from build123d import *

# Parameters (mm, degrees)
SKETCH1_W              = 55
SKETCH1_H              = 20
BOSS_EXTRUDE1_DEPTH    = 25
CHAMFER1_SIZE          = 2
CUT_EXTRUDE1_DEPTH     = 8
HOLE1_D                = 6.6
M12_TAPPED_HOLE1_D     = 10.2
M14X1_5_TAPPED_HOLE1_D = 12.5


with BuildPart() as part:
    # Sketch1 → Boss-Extrude1 (new body)
    with BuildSketch(Plane.XY):
        with Locations((0.549312304, 3.110465116)):
            Rectangle(SKETCH1_W, SKETCH1_H)
    extrude(amount=BOSS_EXTRUDE1_DEPTH)

    # Chamfer1
    chamfer1_edges = [part.edges().sort_by_distance(p)[0] for p in [
        (-26.950687696, 13.110465116, 12.5),
        (28.049312304, 13.110465116, 12.5),
        (28.049312304, -6.889534884, 12.5),
        (-26.950687696, -6.889534884, 12.5),
    ]]
    chamfer(chamfer1_edges, length=CHAMFER1_SIZE)

    # Sketch2 → Cut-Extrude1 (cut)
    with BuildSketch(Plane.XY.offset(25)):
        with BuildLine():
            Line((-21.950687696, 8.610465116), (-26.950687696, 8.610465116))
            Line((-26.950687696, 8.610465116), (-26.950687696, -2.389534884))
            Line((-26.950687696, -2.389534884), (-21.950687696, -2.389534884))
            ThreePointArc((-21.950687696, -2.389534884), (-16.450687696, 3.110465116), (-21.950687696, 8.610465116))
        make_face()
        with BuildLine():
            Line((23.049312304, 8.610465116), (28.049312304, 8.610465116))
            Line((28.049312304, 8.610465116), (28.049312304, -2.389534884))
            Line((28.049312304, -2.389534884), (23.049312304, -2.389534884))
            ThreePointArc((23.049312304, -2.389534884), (17.549312304, 3.110465116), (23.049312304, 8.610465116))
        make_face()
    extrude(amount=-CUT_EXTRUDE1_DEPTH, mode=Mode.SUBTRACT)

    # Hole1 (through all)
    with Locations(Plane.XY.offset(17)):
        with Locations((-21.950687696, 3.110465116), (23.049312304, 3.110465116)):
            Hole(HOLE1_D / 2)

    # M12 Tapped Hole1 (through all)
    with Locations(Plane(origin=(0, -6.889534884, 0), x_dir=(-1, 0, 0), z_dir=(0, -1, 0))):
        with Locations((9.450687696, -12.5)):
            Hole(M12_TAPPED_HOLE1_D / 2)

    # M14x1.5 Tapped Hole1 (through all)
    with Locations(Plane(origin=(0, -6.889534884, 0), x_dir=(-1, 0, 0), z_dir=(0, -1, 0))):
        with Locations((-10.549312304, -12.5)):
            Hole(M14X1_5_TAPPED_HOLE1_D / 2)


solid = part.part
Model file for the job. Use its own axes, mm. A direction names the side the tool comes from. Round coordinates to 2 decimals unless told otherwise and drop trailing zeros. Loops run counter-clockwise (first coordinate to the right, second up) from the corner with the lowest first, then second, coordinate; pieces in that order, holes last. Notation, with made-up numbers: (-22.75, -27.5) - (4.25, -27.5) arc R6 cw to (4.25, -20.5) - close; hole circle Ø10 at (73.5, -28). An arc over 180 degrees is marked (long way). Write each question's results on one line, items separated by ' | '.
(1) Mould opens along Y. For faces 4 (the cylindrical face through (16.323, 3.25, 14.894)), 5 (the flat face through (0, -6.89, 12)), 6 (the flat face through (0, 13.11, 12)), 7 (the cylindrical face through (17.55, 2.99, 21.06)) say: released by +Y, released by -Y, zero draft, split by the parting line, or undercut.
Answer below:
face 4: zero draft | face 5: released by -Y | face 6: released by +Y | face 7: undercut
(2) Wall check: L1, parallel to X at y = 6, z = 11; L2, parallel to X at y = 11, z = 11.5; L3, parallel to X at y = -3, z = 13.75. Give the ranges that are in metal, low to high.
Answer below:
L1: x = -26.95 to -23.54, -20.36 to -14.33, -4.58 to 4.48, 16.62 to 21.46, 24.64 to 28.05 | L2: x = -26.95 to -14.45, -4.45 to 4.38, 16.72 to 28.05 | L3: x = -26.95 to -14.4, -4.51 to 4.43, 16.67 to 28.05
(3) 3-axis set-ups, long thin cutter, end or side, ignore diameter. For faces 1 (the flat face through (25, 6, 17)), 2 (the flat face through (-24, 8.61, 21)), 3 (the flat face through (-25.94, 12.12, 12.32)): which of +Z, -Z, +X, -X, +Y, -Y reach the whole face in a straight line?
Answer below:
face 1: +Z, +X | face 2: +Z, -X | face 3: +Z, -Z, -X, +Y
(4) Saw through at B-B, the plane z = 12.5. List the corners of the cut face in (x, y), then the cut area to 3 significant figures.
Answer below:
outline: (-26.95, -4.89) - (-24.95, -6.89) - (-14.55, -6.89) - (-14.55, 13.11) - (-24.95, 13.11) - (-26.95, 11.11) - close; (-4.35, -6.89) - (4.3, -6.89) - (4.3, 13.11) - (-4.35, 13.11) - close; (16.8, -6.89) - (26.05, -6.89) - (28.05, -4.89) - (28.05, 11.11) - (26.05, 13.11) - (16.8, 13.11) - close; hole circle Ø6.6 at (-21.95, 3.11); hole circle Ø6.6 at (23.05, 3.11) | area: 570 mm^2
(5) Saw through at D-D, the plane x = 6. List the corners of the cut face in (y, z).
Answer below:
outline: (-6.89, 0) - (13.11, 0) - (13.11, 8.21) - (-6.89, 8.21) - close; (-6.89, 16.79) - (13.11, 16.79) - (13.11, 25) - (-6.89, 25) - close
(6) Pin check, flat tips, straight feed: pin 1 (4 mm diameter, centred on x = -21.95, y = 3.11, fed in from +Z); pin 2 (7.5 mm diameter, centred on x = 23.05, y = 3.11, fed in from +Z); pin 3 (2 mm diameter, centred on y = -0.5, z = 20, fed in from +X). Stop position of each tip, or through.
Answer below:
pin 1: passes through | pin 2: stops at z = 17 | pin 3: stops at x = 20.05
(7) Saw through at C-C, the plane y = 9.5. List the corners of the cut face in (x, z).
Answer below:
outline: (-26.95, 0) - (28.05, 0) - (28.05, 25) - (-26.95, 25) - close; hole circle Ø10.2 at (-9.45, 12.5); hole circle Ø12.5 at (10.55, 12.5)
(8) Saw through at A-A, the plane y = 0.5. List the corners of the cut face in (x, z).
Answer below:
outline: (-26.95, 0) - (-23.97, 0) - (-23.97, 17) - (-26.95, 17) - close; (-19.93, 0) - (21.03, 0) - (21.03, 17) - (18.21, 17) - (18.21, 25) - (-17.11, 25) - (-17.11, 17) - (-19.93, 17) - close; (25.07, 0) - (28.05, 0) - (28.05, 17) - (25.07, 17) - close; hole circle Ø10.2 at (-9.45, 12.5); hole circle Ø12.5 at (10.55, 12.5)
